Source: CAD feature listing. Evaluate the final solid. Frame: model axes, mm. Give positions to 0.01 mm unless a question says otherwise; leave off trailing zeros. Order: outer loops, then holes, each group sorted by start corner. A loop starts at its lowest first (then second) coordinate and runs counter-clockwise, first axis right, second up.
```python
from build123d import *

# Parameters (mm, degrees)
SKETCH1_W           = 1290
SKETCH1_H           = 700
BOSS_EXTRUDE1_DEPTH = 20
CUT_EXTRUDE1_DEPTH  = 20
FILLET1_R           = 10


with BuildPart() as part:
    # Sketch1 → Boss-Extrude1 (new body)
    with BuildSketch(Plane.XY):
        Rectangle(SKETCH1_W, SKETCH1_H)
    extrude(amount=BOSS_EXTRUDE1_DEPTH)

    # Sketch2 → Cut-Extrude1 (cut)
    with BuildSketch(Plane.XY.offset(20)):
        with BuildLine():
            Line((-407, 50), (-407, 350))
            Line((-407, 350), (-133, 350))
            Line((-133, 350), (-133, 50))
            ThreePointArc((-133, 50), (-270, -87), (-407, 50))
        make_face()
        with BuildLine():
            Line((407, 350), (133, 350))
            Line((133, 350), (133, 50))
            ThreePointArc((133, 50), (270, -87), (407, 50))
            Line((407, 50), (407, 350))
        make_face()
    extrude(amount=-CUT_EXTRUDE1_DEPTH, mode=Mode.SUBTRACT)

    # Fillet1
    fillet1_edges = [part.edges().sort_by_distance(p)[0] for p in [
        (645, -350, 10),
        (-645, -350, 10),
    ]]
    fillet(fillet1_edges, radius=FILLET1_R)


solid = part.part
```
1) Material intervals for L1, parallel to X at y = 94, z = 4.25; L2, parallel to X at y = 45.5, z = 8.25; L3, parallel to Y at x = 268, z = 6.5, sorted ascending.
Report:
L1: x = -645 to -407, -133 to 133, 407 to 645
L2: x = -645 to -406.93, -133.07 to 133.07, 406.93 to 645
L3: y = -350 to -86.99
2) Section query D-D, the plane y = 6.5. Return the cut outline in (x, z), and give its area (3 significant figures).
Report:
outline: (-645, 0) - (-399.91, 0) - (-399.91, 20) - (-645, 20) - close; (-140.09, 0) - (140.09, 0) - (140.09, 20) - (-140.09, 20) - close; (399.91, 0) - (645, 0) - (645, 20) - (399.91, 20) - close
area: 15,400 mm2
3) Section query C-C, the plane x = 270. Return the cut outline in (y, z), and give its area (3 significant figures).
Report:
outline: (-350, 0) - (-87, 0) - (-87, 20) - (-350, 20) - close
area: 5,260 mm2
4) Section query B-B, the plane z = 10. Return the cut outline in (x, y).
Report:
outline: (-645, -340) arc R10 ccw to (-635, -350) - (635, -350) arc R10 ccw to (645, -340) - (645, 350) - (407, 350) - (407, 50) arc R137 cw to (133, 50) - (133, 350) - (-133, 350) - (-133, 50) arc R137 cw to (-407, 50) - (-407, 350) - (-645, 350) - close
5) Section query A-A, the plane y = 222. Return the cut outline in (x, z).
Report:
outline: (-645, 0) - (-407, 0) - (-407, 20) - (-645, 20) - close; (-133, 0) - (133, 0) - (133, 20) - (-133, 20) - close; (407, 0) - (645, 0) - (645, 20) - (407, 20) - close
6) Draft query along X for faces 1 (the cylindrical face through (266.987, -86.967, 10.14)), 2 (the flat face through (-9, -73, 20)). Return one class per face: +X half, -X half, draft (parallel to the pull), parting line (faces both ways), or undercut.
Report:
face 1: undercut
face 2: draft
